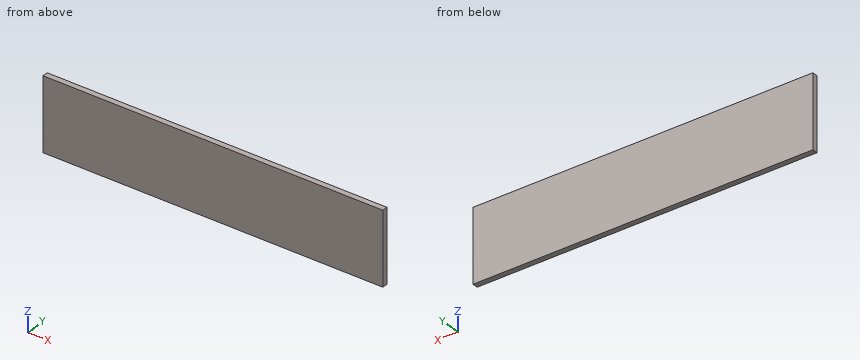
from build123d import *

# Parameters (mm, degrees)
SKETCH_1_W      = 1346
SKETCH_1_H      = 288
EXTRUDE_1_DEPTH = 20
SHELL_1_T       = -2
SKETCH_2_W      = 1346
SKETCH_2_H      = 288
EXTRUDE_2_DEPTH = 2


with BuildPart() as part:
    # 草图1 → 凸台-拉伸1 (new body)
    with BuildSketch(Plane(origin=(0, 0, 0), x_dir=(1, 0, 0), z_dir=(0, 1, 0))):
        Rectangle(SKETCH_1_W, SKETCH_1_H)
    extrude(amount=-EXTRUDE_1_DEPTH)

    # 抽壳1
    shell_1_openings = [part.faces().sort_by_distance(p)[0] for p in [
        (0, -20, 0),
    ]]
    offset(amount=SHELL_1_T, openings=shell_1_openings, kind=Kind.INTERSECTION)

    # 草图2 → 凸台-拉伸2 (add)
    with BuildSketch(Plane.XZ.offset(20)):
        Rectangle(SKETCH_2_W, SKETCH_2_H)
    extrude(amount=EXTRUDE_2_DEPTH)


solid = part.part
The listing builds one solid part. Answer for the finished solid, in the listing's coordinates (mm). Round coordinates to 2 decimals unless told otherwise and drop trailing zeros. Loops run counter-clockwise (first coordinate to the right, second up) from the corner with the lowest first, then second, coordinate; pieces in that order, holes last. Notation, with made-up numbers: M -22.5,36.25 L -10.5,36.25 A6 ccw -10.5,42.25 Z; hole C 27.5,77 d9. An arc over 180 degrees is marked long. Write each question's results on one line, items separated by ' | '. Start each with the question number.
1) Find section B-B on y = -7. Write down the section's boundary in (x, z), plus the area to 3 significant figures.
2) Straight lines are drawn through the part: probe 1 along Z at (x, y) = (-396.5, -5.5); probe 2 along X at (y, z) = (-6.5, -88); probe 3 along Y at (x, z) = (-521, 82). For each, find the intervals that lie inside material, in ascending order.
3) Find section A-A on z = 23.5. Write down the section's boundary in (x, y).
Final values:
1) outline: M -673,-144 L 673,-144 L 673,144 L -673,144 Z; hole M -671,-142 L 671,-142 L 671,142 L -671,142 Z | area: 6,520 mm²
2) probe 1: -144 to -142, 142 to 144 | probe 2: -673 to -671, 671 to 673 | probe 3: -22 to -20, -2 to 0
3) outline: M -673,-22 L 673,-22 L 673,0 L -673,0 Z; hole M -671,-20 L 671,-20 L 671,-2 L -671,-2 Z
